Answer from the drawing. Dimensions are ordinates in mm from the lowest x, y and z of the part. A direction names the side the tool comes from. Coordinates: 2 decimals unless noted, no trailing zeros. Order: outer loops, then holes, each group sorted by start corner. A loop starts at its lowest first (then second) coordinate and runs counter-clockwise, first axis right, second up. Notation, with made-up numbers: M 68.5,-16 L 85.5,-16 A19 cw 85.5,-2 Z; hole C -10.75,-26 d5. An arc over 180 degrees is marked long. Use a Markdown table: item, result.
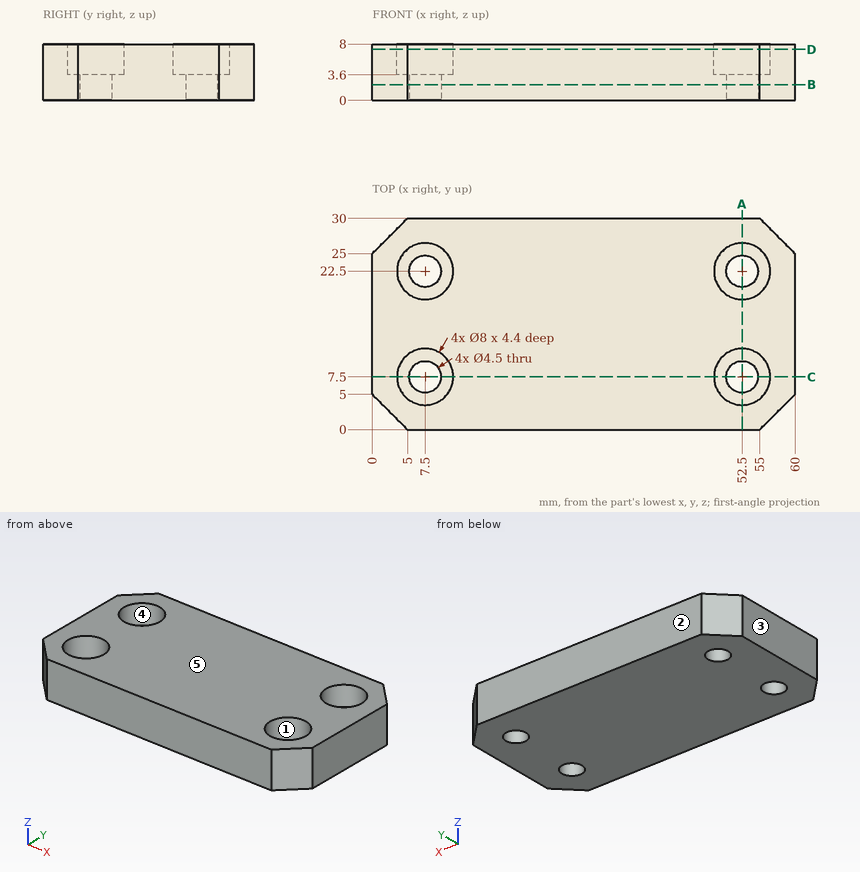
(1) Straight lines are drawn through the part: L1, parallel to Y at x = 7.5, z = 4.65; L2, parallel to Y at x = 52.5, z = 2.75; L3, parallel to X at y = 24, z = 7.75. For each, find the intervals that lie inside material, in ascending order.
Conclusion:
| item | result |
|---|---|
| L1 | 0 to 3.5, 11.5 to 18.5, 26.5 to 30 |
| L2 | 0 to 5.25, 9.75 to 20.25, 24.75 to 30 |
| L3 | 0 to 3.79, 11.21 to 48.79, 56.21 to 60 |
(2) A cutting plane is placed at D-D (z = 7.25). Determine the outline of the cut face in (x, y).
Conclusion:
| item | result |
|---|---|
| outline | M 0,5 L 5,0 L 55,0 L 60,5 L 60,25 L 55,30 L 5,30 L 0,25 Z; hole C 7.5,7.5 d8; hole C 7.5,22.5 d8; hole C 52.5,7.5 d8; hole C 52.5,22.5 d8 |
(3) Determine the mould class of the marked faces 3, 4 and 5 for opening direction X: pulls with the +X half, pulls with the -X half, needs draft (parallel to the pull), parting line crosses it, or undercut.
Conclusion:
| item | result |
|---|---|
| face 3 | pulls with the -X half |
| face 4 | undercut |
| face 5 | needs draft |
(4) A cutting plane is placed at B-B (z = 2.25). Determine the outline of the cut face in (x, y), then the cut area to 3 significant figures.
Conclusion:
| item | result |
|---|---|
| outline | M 0,5 L 5,0 L 55,0 L 60,5 L 60,25 L 55,30 L 5,30 L 0,25 Z; hole C 7.5,7.5 d4.5; hole C 7.5,22.5 d4.5; hole C 52.5,7.5 d4.5; hole C 52.5,22.5 d4.5 |
| area | 1,690 mm2 |
(5) Given P1, Ø2.5, axis at x = 51.5, y = 24, coming from the +Z side; P2, Ø4, axis at x = 52.5, y = 7.5, coming from the -Z side, each flat-ended and moving along its own axis, determine where each tip first touches the part or whether it passes through.
Conclusion:
| item | result |
|---|---|
| P1 | z = 3.6 |
| P2 | through |
(6) A cutting plane is placed at C-C (y = 7.5). Determine the outline of the cut face in (x, z), then the cut area to 3 significant figures.
Conclusion:
| item | result |
|---|---|
| outline | M 0,0 L 5.25,0 L 5.25,3.6 L 3.5,3.6 L 3.5,8 L 0,8 Z; M 9.75,0 L 50.25,0 L 50.25,3.6 L 48.5,3.6 L 48.5,8 L 11.5,8 L 11.5,3.6 L 9.75,3.6 Z; M 54.75,0 L 60,0 L 60,8 L 56.5,8 L 56.5,3.6 L 54.75,3.6 Z |
| area | 377 mm2 |
(7) Which of the six approach directions +Z, -Z, +X, -X, +Y, -Y give full straight-line access (tool end or side, diameter ignored) to the marked faces 1 and 2?
Conclusion:
| item | result |
|---|---|
| face 1 | +Z |
| face 2 | +Z, -Z, +X, -X, +Y |
(8) A cutting plane is placed at A-A (x = 52.5). Determine the outline of the cut face in (y, z).
Conclusion:
| item | result |
|---|---|
| outline | M 0,0 L 5.25,0 L 5.25,3.6 L 3.5,3.6 L 3.5,8 L 0,8 Z; M 9.75,0 L 20.25,0 L 20.25,3.6 L 18.5,3.6 L 18.5,8 L 11.5,8 L 11.5,3.6 L 9.75,3.6 Z; M 24.75,0 L 30,0 L 30,8 L 26.5,8 L 26.5,3.6 L 24.75,3.6 Z |
